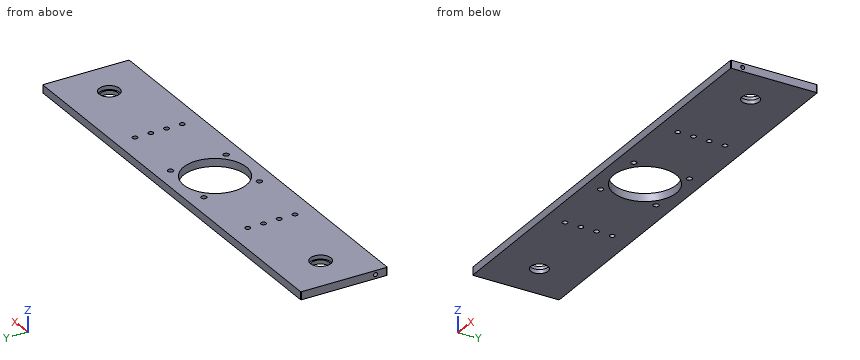
from build123d import *

# Parameters (mm, degrees)
SKETCH1_W           = 550
SKETCH1_H           = 110
BOSS_EXTRUDE1_DEPTH = 10
SKETCH3_R           = 13
CUT_EXTRUDE2_DEPTH  = 5
SKETCH4_R           = 11
CUT_EXTRUDE3_DEPTH  = 281.490641555
SKETCH5_R           = 40
CUT_EXTRUDE4_DEPTH  = 281.624304008
SKETCH6_R           = 3.5
CUT_EXTRUDE5_DEPTH  = 281.624304008
SKETCH7_R           = 3.25
CUT_EXTRUDE6_DEPTH  = 281.624304008
FILLET1_R           = 1


with BuildPart() as part:
    # Sketch1 → Boss-Extrude1 (new body)
    with BuildSketch(Plane.XY):
        Rectangle(SKETCH1_W, SKETCH1_H)
    extrude(amount=BOSS_EXTRUDE1_DEPTH)

    # Sketch3 → Cut-Extrude2 (cut)
    with BuildSketch(Plane.XY.offset(10)):
        with Locations((225, 0)):
            Circle(SKETCH3_R)
        with Locations(Location((-225, 0, 0), (0, 0, 180))):
            Circle(SKETCH3_R)
    extrude(amount=-CUT_EXTRUDE2_DEPTH, mode=Mode.SUBTRACT)

    # Sketch4 → Cut-Extrude3 (cut, through all)
    with BuildSketch(Plane.XY.offset(5)):
        with Locations((225, 0)):
            Circle(SKETCH4_R)
        with Locations(Location((-225, 0, 0), (0, 0, 180))):
            Circle(SKETCH4_R)
    extrude(amount=-CUT_EXTRUDE3_DEPTH, mode=Mode.SUBTRACT)

    # Sketch5 → Cut-Extrude4 (cut, through all)
    with BuildSketch(Plane.XY.offset(10)):
        Circle(SKETCH5_R)
    extrude(amount=-CUT_EXTRUDE4_DEPTH, mode=Mode.SUBTRACT)

    # Sketch6 → Cut-Extrude5 (cut, through all)
    with BuildSketch(Plane.XY.offset(10)):
        with Locations((-35.355339059, 35.355339059)):
            Circle(SKETCH6_R)
        with Locations((35.355339059, 35.355339059)):
            Circle(SKETCH6_R)
        with Locations((35.355339059, -35.355339059)):
            Circle(SKETCH6_R)
        with Locations((-35.355339059, -35.355339059)):
            Circle(SKETCH6_R)
    extrude(amount=-CUT_EXTRUDE5_DEPTH, mode=Mode.SUBTRACT)

    # Sketch7 → Cut-Extrude6 (cut, through all)
    with BuildSketch(Plane.XY.offset(10)):
        with Locations((-120, -10)):
            Circle(SKETCH7_R)
        with Locations((120, -10)):
            Circle(SKETCH7_R)
        with Locations((120, 10)):
            Circle(SKETCH7_R)
        with Locations((-120, 10)):
            Circle(SKETCH7_R)
        with Locations((-120, -30)):
            Circle(SKETCH7_R)
        with Locations((-120, 30)):
            Circle(SKETCH7_R)
        with Locations((120, 30)):
            Circle(SKETCH7_R)
        with Locations((120, -30)):
            Circle(SKETCH7_R)
    extrude(amount=-CUT_EXTRUDE6_DEPTH, mode=Mode.SUBTRACT)

    # Fillet1
    fillet1_edges = [part.edges().sort_by_distance(p)[0] for p in [
        (-275, 55, 5),
        (275, 55, 5),
        (275, -55, 5),
        (-275, -55, 5),
    ]]
    fillet(fillet1_edges, radius=FILLET1_R)

    # Sketch9 → M6 Tapped Hole1 (revolve, cut)
    with BuildSketch(Plane(origin=(-275, -40, 5), x_dir=(0, 0, 1), z_dir=(0, 1, 0))):
        Polygon((0, 0), (0, 19.502151548), (2.5, 18), (2.5, 0), align=None)
    m6_tapped_hole1 = revolve(axis=Axis((-281.35, -40, 5), (1, 0, 0)), mode=Mode.SUBTRACT)

    # Mirror1: M6 Tapped Hole1 across plane
    add(m6_tapped_hole1.mirror(Plane(origin=(0, 0, 0), x_dir=(0, 0, 1), z_dir=(1, 0, 0))), mode=Mode.SUBTRACT)


solid = part.part
Here's how the part is built. I have some questions about the finished solid (model axes, mm). Round coordinates to 2 decimals unless told otherwise and drop trailing zeros. Loops run counter-clockwise (first coordinate to the right, second up) from the corner with the lowest first, then second, coordinate; pieces in that order, holes last. Notation, with made-up numbers: (32, 61.25) -> (64, 61.25) arc R18 ccw to (64, 87.25) -> close; hole circle Ø2 at (-6, 50.5). An arc over 180 degrees is marked (long way). Write each question's results on one line, items separated by ' | '.
(1) If we section it at A-A, the plane x = 0: List the corners of the cut face in (y, z) for me.
Worked answers:
outline: (-55, 0) -> (-40, 0) -> (-40, 10) -> (-55, 10) -> close; (40, 0) -> (55, 0) -> (55, 10) -> (40, 10) -> close
(2) For P1, Ø4, axis at y = -40, z = 5, coming from the +X side, with a flat end and sliding along its axis, tell me the tip position at first contact or that it passes through.
Worked answers:
P1: x = 256.7
(3) If we section it at B-B, the plane y = -20.5: List the corners of the cut face in (x, z) for me, then the cut area to 3 significant figures.
Worked answers:
outline: (-275, 0) -> (-34.35, 0) -> (-34.35, 10) -> (-275, 10) -> close; (34.35, 0) -> (275, 0) -> (275, 10) -> (34.35, 10) -> close | area: 4,810 mm2
(4) If I drill on L1, parallel to Y at x = 120, z = 4.5; L2, parallel to Y at x = -226, z = 7.5; L3, parallel to X at y = -1, z = 2, over which ranges is the centre line in solid material (lowest first)?
Worked answers:
L1: -55 to -33.25, -26.75 to -13.25, -6.75 to 6.75, 13.25 to 26.75, 33.25 to 55 | L2: -55 to -12.96, 12.96 to 55 | L3: -275 to -235.95, -214.05 to -39.99, 39.99 to 214.05, 235.95 to 275
(5) If we section it at C-C, the plane x = -225: List the corners of the cut face in (y, z) for me, then the cut area to 3 significant figures.
Worked answers:
outline: (-55, 0) -> (-11, 0) -> (-11, 5) -> (-13, 5) -> (-13, 10) -> (-55, 10) -> close; (11, 0) -> (55, 0) -> (55, 10) -> (13, 10) -> (13, 5) -> (11, 5) -> close | area: 860 mm2
